```python
from build123d import *

# Parameters (mm, degrees)
SKETCH_1_W               = 15
SKETCH_1_H               = 30
EXTRUDE_1_DEPTH          = 6
SKETCH_2_R               = 0.5
EXTRUDE_2_DEPTH          = 25
PATTERN_LINEAR_1_COUNT   = 4
PATTERN_LINEAR_1_PITCH   = 4
MIRROR_1_COPY_1_SKETCH_R = 0.5
MIRROR_1_COPY_1_DEPTH    = 25
MIRROR_1_COPY_2_SKETCH_R = 0.5
MIRROR_1_COPY_2_DEPTH    = 25
MIRROR_1_COPY_3_SKETCH_R = 0.5
MIRROR_1_COPY_3_DEPTH    = 25
MIRROR_1_COPY_4_SKETCH_R = 0.5
MIRROR_1_COPY_4_DEPTH    = 25


with BuildPart() as part:
    # 草图1 → 凸台-拉伸1 (new, symmetric)
    with BuildSketch(Plane.XY):
        Rectangle(SKETCH_1_W, SKETCH_1_H)
    extrude(amount=EXTRUDE_1_DEPTH, both=True)

    # 草图2 → 凸台-拉伸2 (add)
    with BuildSketch(Plane(origin=(7.5, 0, 0), x_dir=(0, 0, -1), z_dir=(1, 0, 0))):
        with Locations(Location((-4, 0, 0), (0, 0, 180))):
            Circle(SKETCH_2_R)
        with Locations(Location((-2, 0, 0), (0, 0, 180))):
            Circle(SKETCH_2_R)
        with Locations(Location((0, 0, 0), (0, 0, 180))):
            Circle(SKETCH_2_R)
        with Locations(Location((2, 0, 0), (0, 0, 180))):
            Circle(SKETCH_2_R)
        with Locations(Location((4, 0, 0), (0, 0, 180))):
            Circle(SKETCH_2_R)
    extrude_2 = extrude(amount=EXTRUDE_2_DEPTH)

    # 阵列(线性)1: 凸台-拉伸2 ×4
    with Locations(*[(0, -i * PATTERN_LINEAR_1_PITCH, 0) for i in range(1, PATTERN_LINEAR_1_COUNT)]):
        add(extrude_2)

    # 镜向1 copy 1 sketch → 镜向1 copy 1 (add)
    with BuildSketch(Plane(origin=(7.5, 4, 0), x_dir=(0, 0, -1), z_dir=(1, 0, 0))):
        with Locations((-4, 0)):
            Circle(MIRROR_1_COPY_1_SKETCH_R)
        with Locations((-2, 0)):
            Circle(MIRROR_1_COPY_1_SKETCH_R)
        Circle(MIRROR_1_COPY_1_SKETCH_R)
        with Locations((2, 0)):
            Circle(MIRROR_1_COPY_1_SKETCH_R)
        with Locations((4, 0)):
            Circle(MIRROR_1_COPY_1_SKETCH_R)
    extrude(amount=MIRROR_1_COPY_1_DEPTH)

    # 镜向1 copy 2 sketch → 镜向1 copy 2 (add)
    with BuildSketch(Plane(origin=(7.5, 8, 0), x_dir=(0, 0, -1), z_dir=(1, 0, 0))):
        with Locations((-4, 0)):
            Circle(MIRROR_1_COPY_2_SKETCH_R)
        with Locations((-2, 0)):
            Circle(MIRROR_1_COPY_2_SKETCH_R)
        Circle(MIRROR_1_COPY_2_SKETCH_R)
        with Locations((2, 0)):
            Circle(MIRROR_1_COPY_2_SKETCH_R)
        with Locations((4, 0)):
            Circle(MIRROR_1_COPY_2_SKETCH_R)
    extrude(amount=MIRROR_1_COPY_2_DEPTH)

    # 镜向1 copy 3 sketch → 镜向1 copy 3 (add)
    with BuildSketch(Plane(origin=(7.5, 12, 0), x_dir=(0, 0, -1), z_dir=(1, 0, 0))):
        with Locations((-4, 0)):
            Circle(MIRROR_1_COPY_3_SKETCH_R)
        with Locations((-2, 0)):
            Circle(MIRROR_1_COPY_3_SKETCH_R)
        Circle(MIRROR_1_COPY_3_SKETCH_R)
        with Locations((2, 0)):
            Circle(MIRROR_1_COPY_3_SKETCH_R)
        with Locations((4, 0)):
            Circle(MIRROR_1_COPY_3_SKETCH_R)
    extrude(amount=MIRROR_1_COPY_3_DEPTH)

    # 镜向1 copy 4 sketch → 镜向1 copy 4 (add)
    with BuildSketch(Plane(origin=(7.5, 0, 0), x_dir=(0, 0, -1), z_dir=(1, 0, 0))):
        with Locations((-4, 0)):
            Circle(MIRROR_1_COPY_4_SKETCH_R)
        with Locations((-2, 0)):
            Circle(MIRROR_1_COPY_4_SKETCH_R)
        Circle(MIRROR_1_COPY_4_SKETCH_R)
        with Locations((2, 0)):
            Circle(MIRROR_1_COPY_4_SKETCH_R)
        with Locations((4, 0)):
            Circle(MIRROR_1_COPY_4_SKETCH_R)
    extrude(amount=MIRROR_1_COPY_4_DEPTH)


solid = part.part
```
Read the model definition and answer for the solid it produces. Units are mm, in the model's axes. A direction names the side the tool comes from. Coordinates: 2 decimals unless noted, no trailing zeros. Loops run counter-clockwise (first coordinate to the right, second up) from the corner with the lowest first, then second, coordinate; pieces in that order, holes last.
(1) The part is cut by section D-D (z = -3). Determine the outline of the cut face in (x, y).
Solution:
outline: (-7.5, -15) - (7.5, -15) - (7.5, 15) - (-7.5, 15) - close
(2) A tool of negligible diameter and unlimited length cuts with its end or side. For faces 1 (the face through (19.8, 0.3, 3.6)), 2 (the face through (32.5, 4, -2)), from which of +Z, -Z, +X, -X, +Y, -Y can it reach the whole face along a straight path? Write none if from no direction.
Solution:
face 1: +X
face 2: +Z, -Z, +X, +Y, -Y
(3) Flat-ended cylindrical pins translate along their axes: pin 1 Ø5 at (y, z) = (-1.5, -2) entering from +X; pin 2 Ø4 at (x, y) = (13, 6.5) entering from +Z; pin 3 Ø2 at (x, z) = (27, -0.5) entering from +Y. Find the tip coordinate at first contact, or state that the pin passes through.
Solution:
pin 1: stops at x = 32.5
pin 2: stops at z = 4.5
pin 3: stops at y = 12.5
(4) The mould has two halves that part along Z. Classify faces 3 (the face through (19.825, 4.496, -1.935)), 4 (the face through (32.5, -4, 2)): released by +Z, released by -Z, zero draft, split by the parting line, or undercut.
Solution:
face 3: undercut
face 4: zero draft
(5) Consider line 1 along Z through (x, y) = (20, -4); line 2 along X through (y, z) = (-10.25, 5.5). Determine where each line is inside the solid, lowest interval first.
Solution:
line 1: z = -4.5 to -3.5, -2.5 to -1.5, -0.5 to 0.5, 1.5 to 2.5, 3.5 to 4.5
line 2: x = -7.5 to 7.5
(6) The part is cut by section A-A (y = 8). Determine the outline of the cut face in (x, z).
Solution:
outline: (-7.5, -6) - (7.5, -6) - (7.5, -4.5) - (32.5, -4.5) - (32.5, -3.5) - (7.5, -3.5) - (7.5, -2.5) - (32.5, -2.5) - (32.5, -1.5) - (7.5, -1.5) - (7.5, -0.5) - (32.5, -0.5) - (32.5, 0.5) - (7.5, 0.5) - (7.5, 1.5) - (32.5, 1.5) - (32.5, 2.5) - (7.5, 2.5) - (7.5, 3.5) - (32.5, 3.5) - (32.5, 4.5) - (7.5, 4.5) - (7.5, 6) - (-7.5, 6) - close
(7) The part is cut by section C-C (x = 12.5). Count the separate pieces of the cut face and the enclosed holes in it, and give its area (3 significant figures).
Solution:
separate pieces: 35
enclosed holes: 0
area: 27.5 mm2
